Can you work these out from the model? Positions are in its coordinate system, mm. Round coordinates to 2 decimals unless told otherwise and drop trailing zeros. Loops run counter-clockwise (first coordinate to the right, second up) from the corner with the lowest first, then second, coordinate; pieces in that order, holes last. Notation, with made-up numbers: (-35.75, 65.5) -> (17.25, 65.5) arc R23 ccw to (17.25, 75.5) -> close; hole circle Ø11 at (4.5, -20). An arc over 180 degrees is marked (long way). Use a Markdown table: item, result.
from build123d import *

# Parameters (mm, degrees)
SKETCH1_R             = 5
BOSS_EXTRUDE1_DEPTH   = 110
CHAMFER1_SIZE         = 0.5
M4_TAPPED_HOLE1_D     = 3.3
M4_TAPPED_HOLE1_DEPTH = 10.1
M4_TAPPED_HOLE1_TIP   = 0.991420021
M4_TAPPED_HOLE2_D     = 3.3
M4_TAPPED_HOLE2_DEPTH = 10.1
M4_TAPPED_HOLE2_TIP   = 0.991420021


with BuildPart() as part:
    # Sketch1 → Boss-Extrude1 (new, symmetric)
    with BuildSketch(Plane(origin=(0, 0, 0), x_dir=(1, 0, 0), z_dir=(0, 1, 0))):
        with Locations(Location((0, 0, 0), (0, 0, 270))):
            Circle(SKETCH1_R)
    extrude(amount=BOSS_EXTRUDE1_DEPTH, both=True)

    # Chamfer1
    chamfer1_edges = [part.edges().sort_by_distance(p)[0] for p in [
        (0, -110, -5),
        (0, 110, -5),
    ]]
    chamfer(chamfer1_edges, length=CHAMFER1_SIZE)

    # M4 Tapped Hole1
    with Locations(Plane(origin=(0, 110, 0), x_dir=(1, 0, 0), z_dir=(0, 1, 0))):
        with Locations((0, 0)):
            Hole(M4_TAPPED_HOLE1_D / 2, depth=M4_TAPPED_HOLE1_DEPTH)
            with Locations((0, 0, -(M4_TAPPED_HOLE1_DEPTH + M4_TAPPED_HOLE1_TIP / 2))):  # 118° drill point
                Cone(0, M4_TAPPED_HOLE1_D / 2, M4_TAPPED_HOLE1_TIP, mode=Mode.SUBTRACT)

    # M4 Tapped Hole2
    with Locations(Plane(origin=(0, -110, 0), x_dir=(-1, 0, 0), z_dir=(0, -1, 0))):
        with Locations((0, 0)):
            Hole(M4_TAPPED_HOLE2_D / 2, depth=M4_TAPPED_HOLE2_DEPTH)
            with Locations((0, 0, -(M4_TAPPED_HOLE2_DEPTH + M4_TAPPED_HOLE2_TIP / 2))):  # 118° drill point
                Cone(0, M4_TAPPED_HOLE2_D / 2, M4_TAPPED_HOLE2_TIP, mode=Mode.SUBTRACT)


solid = part.part
1. I need wall thicknesses on line 1 (X direction, y = 92, z = 1.75); line 2 (X direction, y = -81, z = -1.25); line 3 (Z direction, x = 4, y = 48). Which ranges of each line are inside material? Lowest first, please.
Answer sheet:
| item | result |
|---|---|
| line 1 | x = -4.68 to 4.68 |
| line 2 | x = -4.84 to 4.84 |
| line 3 | z = -3 to 3 |
2. I want a section at A-A (y = -57.5). Please give me the cut outline in (x, z).
Answer sheet:
| item | result |
|---|---|
| outline | circle Ø10 at (0, 0) |
3. Will these pins go through, and if not, where does the flat tip stop? pin 1 Ø5 at (x, y) = (2.5, -78) entering from +Z; pin 2 Ø2 at (x, y) = (-3, -59.5) entering from +Z; pin 3 Ø1.5 at (x, y) = (2.5, -22) entering from +Z.
Answer sheet:
| item | result |
|---|---|
| pin 1 | stops at z = 5 |
| pin 2 | stops at z = 4.58 |
| pin 3 | stops at z = 4.68 |
